Could you check a few things on this model? Use its own coordinates, in mm. A direction names the side the tool comes from. Give positions to 0.01 mm unless a question says otherwise; leave off trailing zeros. Loops run counter-clockwise (first coordinate to the right, second up) from the corner with the lowest first, then second, coordinate; pieces in that order, holes last. Notation, with made-up numbers: M -13.75,50 L 40.25,50 A26 ccw 40.25,78 Z; hole C 52.25,59 d3. An arc over 180 degrees is marked long. Return JSON: item names as keys, results as strings. Group by question number.
1. If we section it at A-A (y = -33): Write out the boundary of the cut face in (x, z).
2. For pin 1 (8 mm diameter, centred on x = -9, z = 10.5, fed in from -Y), with a flat end and sliding along its axis, tell me the tip position at first contact or that it passes through.
3. Please list where these lines run through material, in increasing order: line 1 (X direction, y = -54.5, z = 4.5); line 2 (Y direction, x = -17, z = 2).
4. If we section it at B-B (z = 17.5): Write out the boundary of the cut face in (x, y).
5. For faces 1 (the flat face through (65, -35, 12)), 2 (the flat face through (-2, 65, 12)), which set-ups out of +Z, -Z, +X, -X, +Y, -Y let a thin tool reach every point of the face, with its end or its side?
6. If we section it at C-C (x = -58): Write out the boundary of the cut face in (y, z).
7. If we mould it in two halves opening along X, with no side actions, what happens to faces 3 (the flat face through (-140, -1, 12)), 4 (the flat face through (1, -5, 12)), 5 (the flat face through (2, 15, 25))? For each: +X half, -X half, draft (parallel to the pull), parting line (faces both ways), or undercut.
```python
from build123d import *

# Parameters (mm, degrees)
BOSS_EXTRUDE1_DEPTH = 25


with BuildPart() as part:
    # Sketch1 → Boss-Extrude1 (new body)
    with BuildSketch(Plane.XY):
        Polygon((-140, 65), (140, 65), (140, -65), (65, -65), (65, -5), (-65, -5), (-65, -65), (-140, -65), align=None)
    extrude(amount=BOSS_EXTRUDE1_DEPTH)


solid = part.part
```
Answer:
{
 "1": {"outline": "M -140,0 L -65,0 L -65,25 L -140,25 Z; M 65,0 L 140,0 L 140,25 L 65,25 Z"},
 "2": {"pin 1": "stops at y = -5"},
 "3": {"line 1": "x = -140 to -65, 65 to 140", "line 2": "y = -5 to 65"},
 "4": {"outline": "M -140,-65 L -65,-65 L -65,-5 L 65,-5 L 65,-65 L 140,-65 L 140,65 L -140,65 Z"},
 "5": {"face 1": "+Z, -Z, -Y", "face 2": "+Z, -Z, +X, -X, +Y"},
 "6": {"outline": "M -5,0 L 65,0 L 65,25 L -5,25 Z"},
 "7": {"face 3": "-X half", "face 4": "undercut", "face 5": "draft"}
}
